from build123d import *

# Parameters (mm, degrees)
BAR_PROFILE_SKETCH_W      = 580
BAR_PROFILE_SKETCH_H      = 80
FLAT_BAR_580X80X16_DEPTH  = 16
HOLE_ROW_SKETCH_R         = 12.6
THROUGH_HOLES_5X_20_DEPTH = 16


with BuildPart() as part:
    # Bar Profile Sketch → Flat Bar 580x80x16 (new body)
    with BuildSketch(Plane.XY):
        Rectangle(BAR_PROFILE_SKETCH_W, BAR_PROFILE_SKETCH_H)
    extrude(amount=FLAT_BAR_580X80X16_DEPTH)

    # Hole Row Sketch → Through Holes 5xØ20 (cut)
    with BuildSketch(Plane.XY.offset(16)):
        with Locations((-240, -20)):
            Circle(HOLE_ROW_SKETCH_R)
        with Locations((-120, -20)):
            Circle(HOLE_ROW_SKETCH_R)
        with Locations((0, -20)):
            Circle(HOLE_ROW_SKETCH_R)
        with Locations((120, -20)):
            Circle(HOLE_ROW_SKETCH_R)
        with Locations((240, -20)):
            Circle(HOLE_ROW_SKETCH_R)
    extrude(amount=-THROUGH_HOLES_5X_20_DEPTH, mode=Mode.SUBTRACT)


solid = part.part
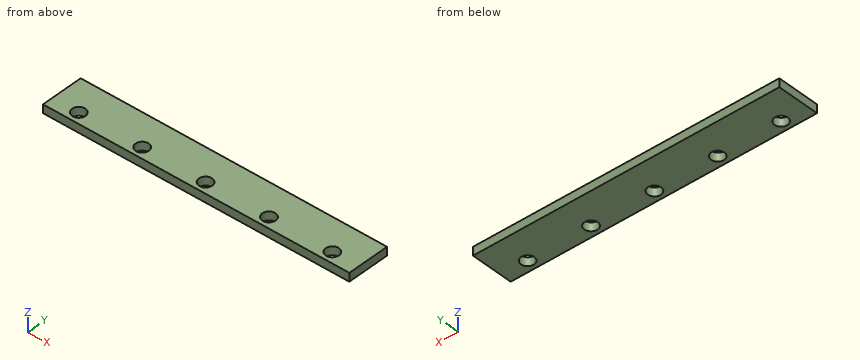
Check sheet for the modelled part. Datum: model origin and axes. Units: mm. Round coordinates to 2 decimals unless told otherwise and drop trailing zeros. Order: outer loops, then holes, each group sorted by start corner. A loop starts at its lowest first (then second) coordinate and runs counter-clockwise, first axis right, second up.
Q1. Cross-section at B-B, the plane y = -20. Enter the section's corners in (x, z).
Filled sheet:
outline: (-290, 0) - (-252.6, 0) - (-252.6, 16) - (-290, 16) - close; (-227.4, 0) - (-132.6, 0) - (-132.6, 16) - (-227.4, 16) - close; (-107.4, 0) - (-12.6, 0) - (-12.6, 16) - (-107.4, 16) - close; (12.6, 0) - (107.4, 0) - (107.4, 16) - (12.6, 16) - close; (132.6, 0) - (227.4, 0) - (227.4, 16) - (132.6, 16) - close; (252.6, 0) - (290, 0) - (290, 16) - (252.6, 16) - close
Q2. Scan lines: L1, parallel to Y at x = -120, z = 6.25; L2, parallel to X at y = -12, z = 12.75; L3, parallel to Y at x = 245, z = 7. Record each from-to range of solid material in increasing order.
Filled sheet:
L1: y = -40 to -32.6, -7.4 to 40
L2: x = -290 to -249.73, -230.27 to -129.73, -110.27 to -9.73, 9.73 to 110.27, 129.73 to 230.27, 249.73 to 290
L3: y = -40 to -31.57, -8.43 to 40
Q3. Cross-section at A-A, the plane x = 120. Enter the section's corners in (y, z).
Filled sheet:
outline: (-40, 0) - (-32.6, 0) - (-32.6, 16) - (-40, 16) - close; (-7.4, 0) - (40, 0) - (40, 16) - (-7.4, 16) - close
